Part model, mm, in its own coordinate system. A direction names the side the tool comes from. Coordinates: 2 decimals unless noted, no trailing zeros. Order: outer loops, then holes, each group sorted by start corner. A loop starts at its lowest first (then second) coordinate and runs counter-clockwise, first axis right, second up.
1) Cut at C-C (x = -1.5). List the corners of the cut face in (y, z).
2) Tool access for faces 4 (the flat face through (5, -39, 1)), 5 (the flat face through (4.37, 21.84, 5.68)), 6 (the cylindrical face through (-2.028, -33.713, -17.535)): list every direction of +Z, -Z, +X, -X, +Y, -Y with a clear straight run to the whole face (end or side of a thin tool).
3) Pin check, flat tips, straight feed: pin 1 Ø11 at (y, z) = (0, -49) entering from -X; pin 2 Ø3 at (x, y) = (10.5, 8.5) entering from -Z; pin 3 Ø8 at (x, y) = (2.5, 41) entering from -Z; pin 4 Ø10 at (x, z) = (11, -46.5) entering from +Y (1 decimal). Stop position of each tip, or through.
4) Cut at D-D (y = -40.5). List the corners of the cut face in (x, z).
5) Cut at A-A (z = -51.5). List the corners of the cut face in (x, y).
6) Mould opens along Z. For faces 1 (the cylindrical face through (9.437, -33.713, -17.535)), 2 (the cylindrical face through (2.535, 0.187, -44.754)), 3 (the flat face through (-5, -16, -16)) say: +Z half, -Z half, draft (parallel to the pull), parting line (faces both ways), or undercut.
7) Wall check: L1, parallel to Y at x = 9.5, z = 0; L2, parallel to Y at x = 3.25, z = 24.5; L3, parallel to X at y = -26.5, z = -39. Give the ranges that are in metal, low to high.
8) Cut at B-B (y = 0). List the corners of the cut face in (x, z), and give its area (3 significant figures).
```python
from build123d import *

# Parameters (mm, degrees)
EXTRUDE_1_DEPTH         = 14
EXTRUDE_1_DEPTH_BACK    = 5
SKETCH_1_R              = 38
SKETCH_2_R              = 60
SKETCH_2_R_2            = 38
EXTRUDE_2_DEPTH         = 5
CHAMFER_1_SIZE          = 1
HOLE_WIZARD_M10_1_D     = 8.5
HOLE_WIZARD_M10_1_DEPTH = 24.5
HOLE_WIZARD_M10_1_TIP   = 2.553657631


with BuildPart() as part:
    # 草图1 → 凸台-拉伸1 (new, two sides: drawn at the far end of the back side and taken through both)
    with BuildSketch(Plane(origin=(0, 0, 0), x_dir=(0, 0, -1), z_dir=(1, 0, 0)).offset(-EXTRUDE_1_DEPTH_BACK)):
        Circle(SKETCH_1_R)
        with BuildLine():
            Line((-4.866153476, 20.428425058), (-6.516153476, 23.28630889))
            Line((-6.516153476, 23.28630889), (-16.908458321, 17.28630889))
            Line((-16.908458321, 17.28630889), (-15.258458321, 14.428425058))
            ThreePointArc((-15.258458321, 14.428425058), (10.5, -18.186533479), (-4.866153476, 20.428425058))
        make_face(mode=Mode.SUBTRACT)
    extrude(amount=EXTRUDE_1_DEPTH + EXTRUDE_1_DEPTH_BACK)

    # 草图2 → 凸台-拉伸2 (add)
    with BuildSketch(Plane(origin=(0, 0, 0), x_dir=(0, 0, -1), z_dir=(1, 0, 0))):
        Circle(SKETCH_2_R)
        Circle(SKETCH_2_R_2, mode=Mode.SUBTRACT)
    extrude(amount=EXTRUDE_2_DEPTH)

    # 倒角1
    chamfer_1_edges = [part.edges().sort_by_distance(p)[0] for p in [
        (-5, 0, 38),
    ]]
    chamfer(chamfer_1_edges, length=CHAMFER_1_SIZE)

    # M10 螺纹孔1
    with Locations(Plane.ZY):
        with Locations((24.5, 42.435244785), (49, 0), (24.5, -42.435244785), (-24.5, -42.435244785), (-49, 0), (-24.5, 42.435244785)):
            Hole(HOLE_WIZARD_M10_1_D / 2, depth=HOLE_WIZARD_M10_1_DEPTH)
            with Locations((0, 0, -(HOLE_WIZARD_M10_1_DEPTH + HOLE_WIZARD_M10_1_TIP / 2))):  # 118° drill point
                Cone(0, HOLE_WIZARD_M10_1_D / 2, HOLE_WIZARD_M10_1_TIP, mode=Mode.SUBTRACT)


solid = part.part
```
Geometry check:
1. outline: circle Ø76 at (0, 0); hole (14.43, 15.26) arc R21 ccw (long way) to (20.43, 4.87) - (23.29, 6.52) - (17.29, 16.91) - close
2. face 4: +X
2. face 5: +X, -X
2. face 6: -X
3. pin 1: stops at x = 0
3. pin 2: stops at z = -37.35
3. pin 3: stops at z = -47.23
3. pin 4: passes through
4. outline: (0, -44.27) - (5, -44.27) - (5, -28.28) - (0, -28.28) - close; (0, -20.72) - (5, -20.72) - (5, 20.72) - (0, 20.72) - close; (0, 28.28) - (5, 28.28) - (5, 44.27) - (0, 44.27) - close
5. outline: (0, -30.79) - (5, -30.79) - (5, -3.44) - (0, -3.44) - close; (0, 3.44) - (5, 3.44) - (5, 30.79) - (0, 30.79) - close
6. face 1: parting line
6. face 2: undercut
6. face 3: draft
7. L1: y = -38 to -21, 21 to 38
7. L2: y = -54.77 to -46.69, -38.19 to 38.19, 46.69 to 54.77
7. L3: x = 0 to 5
8. outline: (-5, -37) - (-4, -38) - (0, -38) - (0, -44.75) - (5, -44.75) - (5, -38) - (14, -38) - (14, -21) - (-5, -21) - close; (-5, 21) - (14, 21) - (14, 38) - (5, 38) - (5, 44.75) - (0, 44.75) - (0, 38) - (-4, 38) - (-5, 37) - close; (0, -60) - (5, -60) - (5, -53.25) - (0, -53.25) - close; (0, 53.25) - (5, 53.25) - (5, 60) - (0, 60) - close
8. area: 780 mm2
